```python
from build123d import *

# Parameters (mm, degrees)
SKETCH_1_W                  = 295
SKETCH_1_H                  = 500
EXTRUDE_1_DEPTH             = 2
HOLE_WIZARD_4_5_4_5_1_D     = 4.5
HOLE_WIZARD_4_5_4_5_1_DEPTH = 8
HOLE_WIZARD_4_5_4_5_1_TIP   = 1.351936393
SKETCH_4_R                  = 10.5
CUT_EXTRUDE_1_DEPTH         = 10


with BuildPart() as part:
    # 草图1 → 凸台-拉伸1 (new body)
    with BuildSketch(Plane.XY):
        Rectangle(SKETCH_1_W, SKETCH_1_H)
    extrude(amount=EXTRUDE_1_DEPTH)

    # Ø4.5 (4.5) 直径孔1
    with Locations(Plane.XY.offset(2)):
        with Locations((-117.5, -240), (-137.5, 0), (-137.5, 200), (-137.5, -200), (-117.5, 240), (32.5, 240), (32.5, -240)):
            Hole(HOLE_WIZARD_4_5_4_5_1_D / 2, depth=HOLE_WIZARD_4_5_4_5_1_DEPTH)
            with Locations((0, 0, -(HOLE_WIZARD_4_5_4_5_1_DEPTH + HOLE_WIZARD_4_5_4_5_1_TIP / 2))):  # 118° drill point
                Cone(0, HOLE_WIZARD_4_5_4_5_1_D / 2, HOLE_WIZARD_4_5_4_5_1_TIP, mode=Mode.SUBTRACT)

    # 草图4 → 切除-拉伸1 (cut)
    with BuildSketch(Plane.XY.offset(2)):
        with Locations((-57.5, 125)):
            Circle(SKETCH_4_R)
        with Locations((-57.5, -125)):
            Circle(SKETCH_4_R)
        with Locations((-57.5, 0)):
            Circle(SKETCH_4_R)
    extrude(amount=-CUT_EXTRUDE_1_DEPTH, mode=Mode.SUBTRACT)


solid = part.part
```
The listing builds one solid part. Answer for the finished solid, in the listing's coordinates (mm). Give positions to 0.01 mm unless a question says otherwise; leave off trailing zeros. Order: outer loops, then holes, each group sorted by start corner. A loop starts at its lowest first (then second) coordinate and runs counter-clockwise, first axis right, second up. Notation, with made-up numbers: (-37, 56.5) -> (-4, 56.5) arc R16 ccw to (-4, 61.5) -> close; hole circle Ø7 at (41.25, 14.5). An arc over 180 degrees is marked (long way). Answer as a JSON object with one key per item and string values. Group by question number.
Item 1: The part is cut by section A-A on y = -125. Write down the section's boundary in (x, z).
Item 2: Determine the mould class of faces 1 (the flat face through (-2, 4, 2)), 2 (the cylindrical face through (-59.78, 114.75, 1.01)) for opening direction X: pulls with the +X half, pulls with the -X half, needs draft (parallel to the pull), parting line crosses it, or undercut.
Item 3: Consider L1, parallel to Y at x = -137.5, z = 0.85; L2, parallel to Y at x = 32.5, z = 1.15; L3, parallel to Y at x = -57, z = 0.85. Determine where each line is inside the solid, lowest interval first. Write a range as from..to.
Item 4: Flat-ended cylindrical pins translate along their axes: pin 1 (5 mm diameter, centred on x = -117.5, y = -240, fed in from -Z); pin 2 (2.5 mm diameter, centred on x = -137.5, y = 0, fed in from -Z). Find the tip coordinate at first contact, or state that the pin passes through.
Item 5: The part is cut by section B-B on x = -61. Write down the section's boundary in (y, z), and give its area (3 significant figures).
Result set:
{
 "1": {"outline": "(-147.5, 0) -> (-68, 0) -> (-68, 2) -> (-147.5, 2) -> close; (-47, 0) -> (147.5, 0) -> (147.5, 2) -> (-47, 2) -> close"},
 "2": {"face 1": "needs draft", "face 2": "undercut"},
 "3": {"L1": "-250..-202.25, -197.75..-2.25, 2.25..197.75, 202.25..250", "L2": "-250..-242.25, -237.75..237.75, 242.25..250", "L3": "-250..-135.49, -114.51..-10.49, 10.49..114.51, 135.49..250"},
 "4": {"pin 1": "z = 0", "pin 2": "through"},
 "5": {"outline": "(-250, 0) -> (-134.9, 0) -> (-134.9, 2) -> (-250, 2) -> close; (-115.1, 0) -> (-9.9, 0) -> (-9.9, 2) -> (-115.1, 2) -> close; (9.9, 0) -> (115.1, 0) -> (115.1, 2) -> (9.9, 2) -> close; (134.9, 0) -> (250, 0) -> (250, 2) -> (134.9, 2) -> close", "area": "881 mm²"}
}
